from build123d import *

# Parameters (mm, degrees)
SKETCH_1_R              = 44.5
EXTRUDE_1_DEPTH         = 976
SKETCH_2_R              = 10
EXTRUDE_2_DEPTH         = 8
EXTRUDE_START           = 8
SKETCH_3_R              = 10
EXTRUDE_3_DEPTH         = 8
HOLE_WIZARD_M10_1_D     = 8.5
HOLE_WIZARD_M10_1_DEPTH = 22.5
HOLE_WIZARD_M10_1_TIP   = 2.553657631
HOLE_WIZARD_M10_2_D     = 8.5
HOLE_WIZARD_M10_2_DEPTH = 22.5
HOLE_WIZARD_M10_2_TIP   = 2.553657631
SKETCH_11_R             = 7.5
CUT_EXTRUDE_1_DEPTH     = 488


with BuildPart() as part:
    # 草图1 → 凸台-拉伸1 (new body)
    with BuildSketch(Plane.XY):
        with Locations(Location((0, 0, 0), (0, 0, 180))):
            Circle(SKETCH_1_R)
    extrude(amount=EXTRUDE_1_DEPTH)

    # 草图2 → 凸台-拉伸2 (add)
    with BuildSketch(Plane.XY.offset(976)):
        Circle(SKETCH_2_R)
    extrude(amount=EXTRUDE_2_DEPTH)

    # 草图3 → 凸台-拉伸3 (add)
    with BuildSketch(Plane(origin=(0, 0, 0), x_dir=(-1, 0, 0), z_dir=(0, 0, -1)).offset(EXTRUDE_START)):
        with Locations(Location((0, 0, 0), (0, 0, 180))):
            Circle(SKETCH_3_R)
    extrude(amount=-EXTRUDE_3_DEPTH)

    # M10 螺纹孔1
    with Locations(Plane(origin=(0, 0, -8), x_dir=(-1, 0, 0), z_dir=(0, 0, -1))):
        with Locations((0, 0)):
            Hole(HOLE_WIZARD_M10_1_D / 2, depth=HOLE_WIZARD_M10_1_DEPTH)
            with Locations((0, 0, -(HOLE_WIZARD_M10_1_DEPTH + HOLE_WIZARD_M10_1_TIP / 2))):  # 118° drill point
                Cone(0, HOLE_WIZARD_M10_1_D / 2, HOLE_WIZARD_M10_1_TIP, mode=Mode.SUBTRACT)

    # M10 螺纹孔2
    with Locations(Plane.XY.offset(984)):
        with Locations((0, 0)):
            Hole(HOLE_WIZARD_M10_2_D / 2, depth=HOLE_WIZARD_M10_2_DEPTH)
            with Locations((0, 0, -(HOLE_WIZARD_M10_2_DEPTH + HOLE_WIZARD_M10_2_TIP / 2))):  # 118° drill point
                Cone(0, HOLE_WIZARD_M10_2_D / 2, HOLE_WIZARD_M10_2_TIP, mode=Mode.SUBTRACT)

    # 草图11 → 切除-拉伸1 (cut, symmetric)
    with BuildSketch(Plane.XY.offset(488)):
        Circle(SKETCH_11_R)
    extrude(amount=CUT_EXTRUDE_1_DEPTH, both=True, mode=Mode.SUBTRACT)


solid = part.part
The model under review builds one solid part; all positions refer to its coordinate system, in mm. A direction names the side the tool comes from. Give positions to 0.01 mm unless a question says otherwise; leave off trailing zeros. Loops run counter-clockwise (first coordinate to the right, second up) from the corner with the lowest first, then second, coordinate; pieces in that order, holes last. Notation, with made-up numbers: (8, 5.5) -> (48, 5.5) arc R21 cw to (48, 30.5) -> close; hole circle Ø3 at (44.5, 2.5). An arc over 180 degrees is marked (long way). Answer as a JSON object with one key per item and string values. Group by question number.
Q1. Take a section at B-B (y = 26.5). Write out the cut boundary in (x, z).
Q2. Tool access review of faces 1 (the cylindrical face through (-7.493, 0.33, 494.832)), 2 (the flat face through (2, 4, -8)), 3 (the flat face through (2, -4, 984)), 4 (the cylindrical face through (-10, 0, -4)), 5 (the cylindrical face through (-2.17, -9.76, 979.94)): name each direction out of +Z, -Z, +X, -X, +Y, -Y from which nothing blocks a thin tool from reaching the whole face with its end or side.
Q3. Insertion check: pin 1 (3 mm diameter, centred on x = 5.5, z = 476, fed in from +Y); pin 2 (8 mm diameter, centred on x = -8.5, y = 33.5, fed in from -Z); pin 3 (1 mm diameter, centred on x = -11.5, y = 28.5, fed in from +Z). Each pin has a flat end and moves straight along its axis. Give the tip position at first contact, or say it passes through.
Q4. Take a section at C-C (x = 29). Write out the cut boundary in (y, z), plus the area to 3 significant figures.
Q5. Wall thickness on line 1 along Y through (x, z) = (0, 980.5); line 2 along Y through (x, z) = (0, 675.5); line 3 along Z through (x, y) = (17, 37): over which ranges is each line inside the solid? List them lowest first.
Q6. Draft analysis for pull direction X (two halves, no side actions). For faces 6 (the flat face through (1, -11, 0)), 7 (the flat face through (3.2, -3.2, 0)), 8 (the cylindrical face through (32.798, -30.075, 481.168)), state which applies: pulls with the +X half, pulls with the -X half, needs draft (parallel to the pull), parting line crosses it, or undercut.
Q7. Take a section at A-A (z = 418). Write out the cut boundary in (x, y), plus the area to 3 significant figures.
Answer below:
{
 "1": {"outline": "(-35.75, 0) -> (35.75, 0) -> (35.75, 976) -> (-35.75, 976) -> close"},
 "2": {"face 1": "none", "face 2": "-Z, +X, -X, +Y, -Y", "face 3": "+Z, +X, -X, +Y, -Y", "face 4": "-Z", "face 5": "+Z"},
 "3": {"pin 1": "stops at y = 44.32", "pin 2": "stops at z = 0", "pin 3": "stops at z = 976"},
 "4": {"outline": "(-33.75, 0) -> (33.75, 0) -> (33.75, 976) -> (-33.75, 976) -> close", "area": "65,900 mm2"},
 "5": {"line 1": "y = -10 to -4.25, 4.25 to 10", "line 2": "y = -44.5 to -7.5, 7.5 to 44.5", "line 3": "z = 0 to 976"},
 "6": {"face 6": "needs draft", "face 7": "undercut", "face 8": "parting line crosses it"},
 "7": {"outline": "circle Ø89 at (0, 0); hole circle Ø15 at (0, 0)", "area": "6,040 mm2"}
}
